Design review of the part built by this model. Coordinates are the model's own, in mm. Face numbers are marked on the shaded views. A direction names the side the tool comes from. Give positions to 0.01 mm unless a question says otherwise; leave off trailing zeros. Write each loop counter-clockwise with the first axis right and the second up, starting at its lowest first coordinate (ties: lowest second). Pieces come first, ordered by that corner, then holes. Notation, with made-up numbers: M 77,-15 L 90,-15 A22 cw 90,-1 Z; hole C 75.25,43.5 d2. An arc over 180 degrees is marked long. One line per item, written item: value. Start each with the question number.
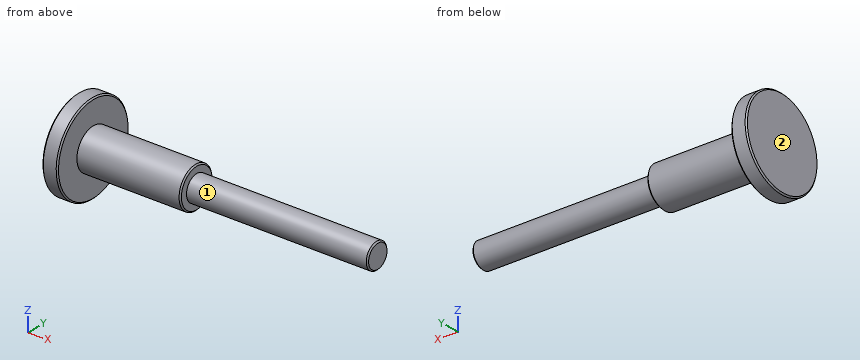
```python
from build123d import *

# Parameters (mm, degrees)
CHAMFER1_SIZE = 0.5
CHAMFER2_SIZE = 0.5


with BuildPart() as part:
    # Sketch1 → Revolve1 (revolve)
    with BuildSketch(Plane.XY, mode=Mode.PRIVATE) as revolve1_sk:
        Polygon((0, 0), (0, 17.5), (6, 17.5), (6, 8), (46, 8), (46, 5), (116, 5), (116, 0), align=None)
    revolve(revolve1_sk.sketch.rotate(Axis((0, 0, 0), (1, 0, 0)), 90), axis=Axis((0, 0, 0), (1, 0, 0)))

    # Chamfer1
    chamfer1_edges = [part.edges().sort_by_distance(p)[0] for p in [
        (46, 0, -8),
        (6, 0, -17.5),
        (0, 0, -17.5),
    ]]
    chamfer(chamfer1_edges, length=CHAMFER1_SIZE)

    # Chamfer2
    chamfer2_edges = [part.edges().sort_by_distance(p)[0] for p in [
        (116, 0, -5),
    ]]
    chamfer(chamfer2_edges, length=CHAMFER2_SIZE)


solid = part.part
```
Q1. Machinability: for the marked faces 1 and 2, which of the approach directions +Z, -Z, +X, -X, +Y, -Y give a long, thin tool a straight path to every point of the face, cutting with its end or side? Answer none if there is none.
Q2. Wall thickness on line 1 (Y direction, x = 66.5, z = -0.5); line 2 (X direction, y = 15, z = 6); line 3 (Y direction, x = 39.5, z = 0): over which ranges is each line inside the solid? List them lowest first. Write a range as from..to.
Q3. For P1, Ø12, axis at x = 15, z = -7.5, coming from the +Y side; P2, Ø3, axis at y = 5.5, z = -10, coming from the +X side, all flat-tipped, find the tip position at first contact; note any pin that passes through.
Q4. Take a section at A-A, the plane y = 0. Give the boundary of the cut face in (x, z).
Q5. Take a section at C-C, the plane x = 105. Give the boundary of the cut face in (y, z).
Q6. Take a section at D-D, the plane x = 26. Give the boundary of the cut face in (y, z), then the cut area to 3 significant figures.
Results list:
1. face 1: +X
1. face 2: +Z, -Z, -X, +Y, -Y
2. line 1: y = -4.97..4.97
2. line 2: x = 0..6
2. line 3: y = -8..8
3. P1: stops at y = 7.86
3. P2: stops at x = 6
4. outline: M 0,-17 L 0.5,-17.5 L 5.5,-17.5 L 6,-17 L 6,-8 L 45.5,-8 L 46,-7.5 L 46,-5 L 115.5,-5 L 116,-4.5 L 116,4.5 L 115.5,5 L 46,5 L 46,7.5 L 45.5,8 L 6,8 L 6,17 L 5.5,17.5 L 0.5,17.5 L 0,17 Z
5. outline: C 0,0 d10
6. outline: C 0,0 d16
6. area: 201 mm^2
